The figure shows three views and two pictorial views of one solid part (mm, origin at its lowest corner). Answer the questions. Give positions to 0.01 mm unless a question says otherwise; leave off trailing zeros. Loops run counter-clockwise (first coordinate to the right, second up) from the corner with the lowest first, then second, coordinate; pieces in that order, holes last. Notation, with made-up numbers: M 2,58 L 33,58 A33 ccw 33,95 Z; hole C 46.25,40.5 d10. An arc over 180 degrees is marked long. Answer in a Markdown table with one row per item. Add a question column.
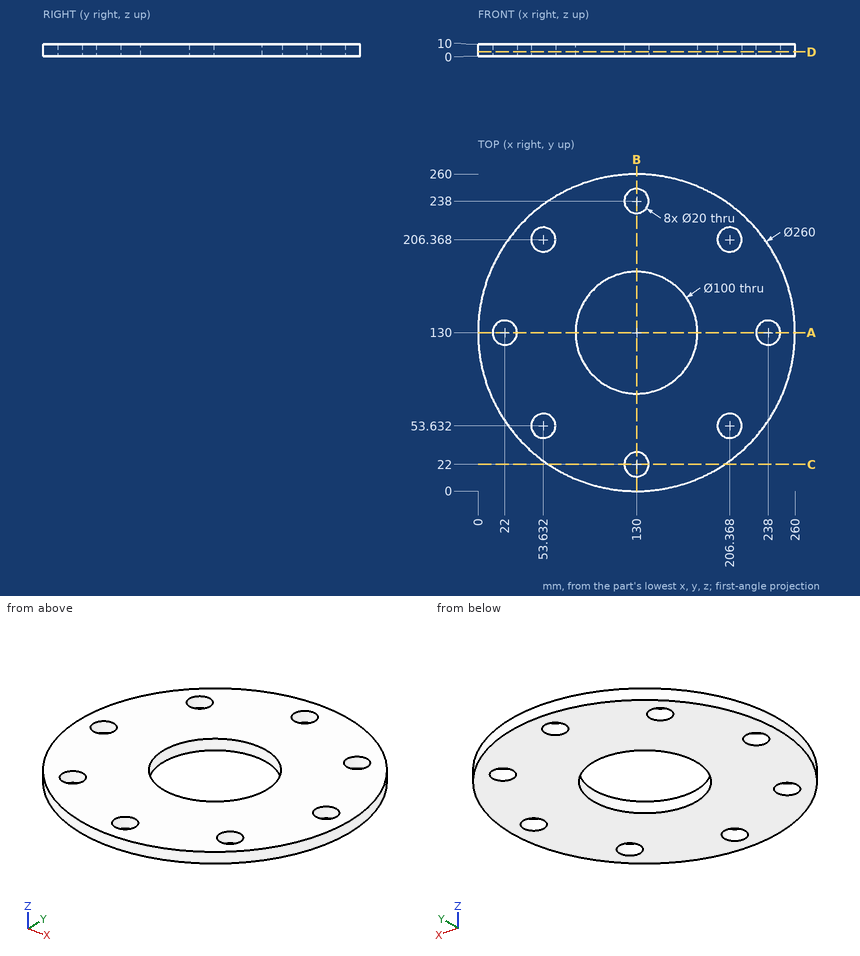
(1) Section D-D, the plane z = 3.5 is taken. State how many separate pieces and enclosed holes the cut face has, and give its area (3 significant figures).
(2) Consider line 1 along X through (y, z) = (200.5, 4.5) (1 decimal); line 2 along Y through (x, z) = (122, 3.75) (1 decimal); line 3 along X through (y, z) = (62, 1.75) (1 decimal). Determine where each line is inside the solid, lowest interval first. Write a range as from..to.
(3) Section C-C, the plane y = 22 is taken. Determine the outline of the cut face in (x, z).
(4) Each of these flat-tipped pins is pushed along its axis until it touches: P1, Ø1.5, axis at x = 100, z = 2, coming from the +Y side; P2, Ø18, axis at x = 130, y = 22, coming from the +Z side; P3, Ø4, axis at y = 229.5, z = 1.5, coming from the -X side (1 decimal); P4, Ø3, axis at x = 190, z = 4, coming from the -Y side. Where does it stop, or does it pass through?
(5) Section A-A, the plane y = 130 is taken. Determine the outline of the cut face in (x, z), and give its area (3 significant figures).
Numbers:
| question | item | result |
|---|---|---|
| 1 | separate pieces | 1 |
| 1 | enclosed holes | 9 |
| 1 | area | 42,700 mm² |
| 2 | line 1 | x = 20.8..45.5, 61.7..198.3, 214.5..239.2 |
| 2 | line 2 | y = 0.2..16, 28..80.6, 179.4..232, 244..259.8 |
| 2 | line 3 | x = 19.2..48.2, 59.1..200.9, 211.8..240.8 |
| 3 | outline | M 57.64,0 L 120,0 L 120,10 L 57.64,10 Z; M 140,0 L 202.36,0 L 202.36,10 L 140,10 Z |
| 4 | P1 | stops at y = 256.67 |
| 4 | P2 | passes through |
| 4 | P3 | stops at x = 44 |
| 4 | P4 | stops at y = 13.91 |
| 5 | outline | M 0,0 L 12,0 L 12,10 L 0,10 Z; M 32,0 L 80,0 L 80,10 L 32,10 Z; M 180,0 L 228,0 L 228,10 L 180,10 Z; M 248,0 L 260,0 L 260,10 L 248,10 Z |
| 5 | area | 1,200 mm² |
